Here's how the part is built. I have some questions about the finished solid (model axes, mm). A direction names the side the tool comes from. Give positions to 0.01 mm unless a question says otherwise; leave off trailing zeros. Write each loop counter-clockwise with the first axis right and the second up, starting at its lowest first coordinate (ties: lowest second). Pieces come first, ordered by that corner, then holes. Notation, with made-up numbers: (-32, -24) -> (3, -24) arc R17 cw to (3, -2) -> close; hole circle Ø5 at (-7.75, 36.25). An arc over 180 degrees is marked (long way). Use one line per item in the form item = value.
```python
from build123d import *

# Parameters (mm, degrees)
SKETCH_1_W          = 20
SKETCH_1_H          = 11
EXTRUDE_1_DEPTH     = 9.5
SKETCH_2_W          = 16.2
SKETCH_2_H          = 29.89512134
CUT_EXTRUDE_1_DEPTH = 2.2
CUT_EXTRUDE_2_DEPTH = 23.814469093


with BuildPart() as part:
    # 草图1 → 凸台-拉伸1 (new body)
    with BuildSketch(Plane.XY):
        Rectangle(SKETCH_1_W, SKETCH_1_H)
    extrude(amount=EXTRUDE_1_DEPTH)

    # 草图2 → 切除-拉伸1 (cut)
    with BuildSketch(Plane.XY.offset(9.5)):
        Rectangle(SKETCH_2_W, SKETCH_2_H)
    extrude(amount=-CUT_EXTRUDE_1_DEPTH, mode=Mode.SUBTRACT)

    # 草图3 → 切除-拉伸2 (cut, through all)
    with BuildSketch(Plane.ZY.offset(10)):
        Polygon((0, 5.5), (3.5, 5.5), (0, 2), align=None)
    cut_extrude_2 = extrude(amount=-CUT_EXTRUDE_2_DEPTH, mode=Mode.SUBTRACT)

    # 镜向1: 切除-拉伸2 across plane
    add(cut_extrude_2.mirror(Plane.ZX), mode=Mode.SUBTRACT)


solid = part.part
```
Q1. I want a section at D-D, the plane z = 1.5. Write out the boundary of the cut face in (x, y), and give its area (3 significant figures).
Result set:
outline = (-10, -3.5) -> (10, -3.5) -> (10, 3.5) -> (-10, 3.5) -> close
area = 140 mm2
Q2. If I drill on line 1 along X through (y, z) = (0.5, 9); line 2 along Z through (x, y) = (1.5, 0.5); line 3 along Y through (x, z) = (6, 1.5), over which ranges is the centre line in solid material (lowest first)? Write a range as from..to.
Result set:
line_1 = -10..-8.1, 8.1..10
line_2 = 0..7.3
line_3 = -3.5..3.5
Q3. If we mould it in two halves opening along X, with no side actions, what happens to faces 1 (the face through (0, 4, 2)), 2 (the face through (-10, 0, 6)), 3 (the face through (8.1, 0, 8))? For each: +X half, -X half, draft (parallel to the pull), parting line (faces both ways), or undercut.
Result set:
face_1 = draft
face_2 = -X half
face_3 = undercut
Q4. I want a section at A-A, the plane z = 8.5. Write out the boundary of the cut face in (x, y).
Result set:
outline = (-10, -5.5) -> (-8.1, -5.5) -> (-8.1, 5.5) -> (-10, 5.5) -> close; (8.1, -5.5) -> (10, -5.5) -> (10, 5.5) -> (8.1, 5.5) -> close
Q5. Which directions (+Z, -Z, +X, -X, +Y, -Y) give clear straight access to the entire face, cutting with the end or side of a thin tool? Please do faces 4 (the face through (0, 5.5, 6)), 5 (the face through (-8.1, 0, 8)).
Result set:
face_4 = +Z, -Z, +X, -X, +Y
face_5 = +Z, +Y, -Y
Q6. I want a section at B-B, the plane x = 6.25. Write out the boundary of the cut face in (y, z), and give its area (4 significant figures).
Result set:
outline = (-5.5, 3.5) -> (-2, 0) -> (2, 0) -> (5.5, 3.5) -> (5.5, 7.3) -> (-5.5, 7.3) -> close
area = 68.05 mm2
Q7. I want a section at C-C, the plane y = -3.5. Write out the boundary of the cut face in (x, z), and give its area (3 significant figures).
Result set:
outline = (-10, 1.5) -> (10, 1.5) -> (10, 9.5) -> (8.1, 9.5) -> (8.1, 7.3) -> (-8.1, 7.3) -> (-8.1, 9.5) -> (-10, 9.5) -> close
area = 124 mm2
Q8. Will these pins go through, and if not, where does the flat tip stop? pin 1 Ø5 at (x, y) = (-6.5, 0.5) entering from +Z; pin 2 Ø3 at (x, z) = (-1.5, 1.5) entering from -Y; pin 3 Ø2 at (x, z) = (-5.5, 1.5) entering from -Y.
Result set:
pin_1 = 9.5
pin_2 = -5
pin_3 = -4.5
